For this review, take the finished solid that the model builds, in its own axes (mm). A direction names the side the tool comes from. Round coordinates to 2 decimals unless told otherwise and drop trailing zeros. Order: outer loops, then holes, each group sorted by start corner. A loop starts at its lowest first (then second) coordinate and runs counter-clockwise, first axis right, second up.
```python
from build123d import *

# Parameters (mm, degrees)
SKETCH1_R                = 5
BOSS_EXTRUDE1_DEPTH      = 3
SKETCH2_R                = 6.5
BOSS_EXTRUDE2_DEPTH      = 4
BOSS_EXTRUDE3_DEPTH      = 2
BOSS_EXTRUDE3_DEPTH_BACK = 1
SKETCH3_R                = 8.5
SKETCH3_R_2              = 6.5
SKETCH4_R                = 5
BOSS_EXTRUDE4_DEPTH      = 9
SKETCH5_R                = 6
BOSS_EXTRUDE5_DEPTH      = 2
SKETCH7_R                = 5
BOSS_EXTRUDE6_DEPTH      = 4
BOSS_EXTRUDE7_START      = 3
SKETCH8_R                = 6.5
BOSS_EXTRUDE7_DEPTH      = 3
SKETCH10_R               = 4.5
BOSS_EXTRUDE8_DEPTH      = 13
DOME1_FACE_RADIUS        = 4.5
DOME1_HEIGHT             = 5
SKETCH11_R               = 1
CUT_EXTRUDE1_DEPTH       = 26


with BuildPart() as part:
    # Sketch1 → Boss-Extrude1 (new body)
    with BuildSketch(Plane.XY):
        with Locations((3, 0)):
            Circle(SKETCH1_R)
    extrude(amount=-BOSS_EXTRUDE1_DEPTH)

    # Sketch2 → Boss-Extrude2 (add)
    with BuildSketch(Plane.XY):
        with Locations((3, 0)):
            Circle(SKETCH2_R)
    extrude(amount=BOSS_EXTRUDE2_DEPTH)

    # Sketch3 → Boss-Extrude3 (add, two sides: drawn at the far end of the back side and taken through both)
    with BuildSketch(Plane.XY.offset(4).offset(-BOSS_EXTRUDE3_DEPTH_BACK)):
        with Locations((3, 0)):
            Circle(SKETCH3_R)
        with Locations((3, 0)):
            Circle(SKETCH3_R_2, mode=Mode.SUBTRACT)
    extrude(amount=BOSS_EXTRUDE3_DEPTH + BOSS_EXTRUDE3_DEPTH_BACK)

    # Sketch4 → Boss-Extrude4 (add)
    with BuildSketch(Plane(origin=(0, 0, -3), x_dir=(-1, 0, 0), z_dir=(0, 0, -1))):
        with Locations(Location((-3, 0, 0), (0, 0, 180))):
            Circle(SKETCH4_R)
    extrude(amount=BOSS_EXTRUDE4_DEPTH)

    # Sketch5 → Boss-Extrude5 (add)
    with BuildSketch(Plane(origin=(0, 0, -12), x_dir=(-1, 0, 0), z_dir=(0, 0, -1))):
        with Locations((-3, 0)):
            Circle(SKETCH5_R)
    extrude(amount=-BOSS_EXTRUDE5_DEPTH)

    # Sketch7 → Boss-Extrude6 (add)
    with BuildSketch(Plane(origin=(0, 0, -12), x_dir=(-1, 0, 0), z_dir=(0, 0, -1))):
        with Locations(Location((-3, 0, 0), (0, 0, 180))):
            Circle(SKETCH7_R)
    extrude(amount=BOSS_EXTRUDE6_DEPTH)

    # Sketch8 → Boss-Extrude7 (add)
    with BuildSketch(Plane(origin=(0, 0, -16), x_dir=(-1, 0, 0), z_dir=(0, 0, -1)).offset(BOSS_EXTRUDE7_START)):
        with Locations(Location((-3, 0, 0), (0, 0, 180))):
            Circle(SKETCH8_R)
    extrude(amount=-BOSS_EXTRUDE7_DEPTH)

    # Sketch10 → Boss-Extrude8 (add)
    with BuildSketch(Plane(origin=(0, 0, -19), x_dir=(-1, 0, 0), z_dir=(0, 0, -1))):
        with Locations((-3, 0)):
            Circle(SKETCH10_R)
    extrude(amount=BOSS_EXTRUDE8_DEPTH)

    # Dome1: a dome of height H over a round flat face of radius A is a cap of a sphere of radius (A * A + H * H) / (2 * H)
    dome1_r = (DOME1_FACE_RADIUS * DOME1_FACE_RADIUS + DOME1_HEIGHT * DOME1_HEIGHT) / (2 * DOME1_HEIGHT)
    dome1_base = Plane((3, 0, -32), z_dir=(0, 0, -1))
    with Locations(dome1_base.offset(DOME1_HEIGHT - dome1_r)):
        dome1_ball = Sphere(dome1_r, mode=Mode.PRIVATE)
    add(split(dome1_ball, bisect_by=dome1_base, keep=Keep.TOP, mode=Mode.PRIVATE))

    # Sketch11 → Cut-Extrude1 (cut)
    with BuildSketch(Plane(origin=(0, 0, -19), x_dir=(-1, 0, 0), z_dir=(0, 0, -1))):
        with Locations(Location((-3, 0, 0), (0, 0, 180))):
            Circle(SKETCH11_R)
    extrude(amount=CUT_EXTRUDE1_DEPTH, mode=Mode.SUBTRACT)


solid = part.part
```
Q1. Mouldability with a two-part tool opening along Y and no side actions: class faces 1 (the face through (-3.265, 5.745, 4.479)), 2 (the face through (1.591, -6.345, 4.986)), 3 (the face through (7, 4, -10)), 4 (the face through (3, 0, 4)) as +Y half, -Y half, draft (parallel to the pull), parting line (faces both ways), or undercut.
Q2. Take a section at D-D, the plane z = -6.5. State the section outline as (x, y) points.
Q3. Take a section at A-A, the plane y = 5.5. State the section outline as (x, z) points, plus the area to 3 significant figures.
Q4. Wall thickness on line 1 (Z direction, x = 6, y = -5); line 2 (Y direction, x = 3, z = -26.25); line 3 (Y direction, x = 3, z = 5.55): over which ranges is each line inside the solid? List them lowest first.
Q5. Take a section at B-B, the plane z = -24.5. State the section outline as (x, y) points, plus the area to 3 significant figures.
Q6. Tool access review of faces 5 (the face through (7.4, -5, 6)), 6 (the face through (7, 4, -12)), 7 (the face through (2.2, 0.6, -27.8)): name each direction out of +Z, -Z, +X, -X, +Y, -Y from which nothing blocks a thin tool from reaching the whole face with its end or side.
Q7. Clearance check with flat-ended pins moving along their axes: pin 1 (3 mm diameter, centred on y = 2, z = -2.5, fed in from +X); pin 2 (8 mm diameter, centred on y = 4, z = -21, fed in from +X); pin 3 (2 mm diameter, centred on x = 10, z = -22, fed in from +Y); pin 4 (9.5 mm diameter, centred on x = 3.5, y = 1.5, fed in from +Z). State where each tip first meets the part, or that it passes through.
Working result:
1. face 1: parting line
1. face 2: undercut
1. face 3: draft
1. face 4: undercut
2. outline: circle Ø10 at (3, 0)
3. outline: (-3.48, 3) - (-0.46, 3) - (-0.46, 0) - (6.46, 0) - (6.46, 3) - (9.48, 3) - (9.48, 6) - (6.46, 6) - (6.46, 4) - (-0.46, 4) - (-0.46, 6) - (-3.48, 6) - close; (-0.46, -19) - (6.46, -19) - (6.46, -16) - (-0.46, -16) - close; (0.6, -12) - (5.4, -12) - (5.4, -10) - (0.6, -10) - close
3. area: 76.2 mm2
4. line 1: z = -19 to -16, -12 to -10, 0 to 4
4. line 2: y = -4.5 to -1, 1 to 4.5
4. line 3: y = -8.5 to -6.5, 6.5 to 8.5
5. outline: circle Ø9 at (3, 0); hole circle Ø2 at (3, 0)
5. area: 60.5 mm2
6. face 5: +Z, +X, -X, +Y, -Y
6. face 6: none
6. face 7: -Z
7. pin 1: stops at x = 7.97
7. pin 2: stops at x = 9.48
7. pin 3: passes through
7. pin 4: stops at z = 4
